Verification items for the finished model (mm, model axes). A direction names the side the tool comes from. Coordinates: 2 decimals unless noted, no trailing zeros. Order: outer loops, then holes, each group sorted by start corner. A loop starts at its lowest first (then second) coordinate and runs counter-clockwise, first axis right, second up. Notation, with made-up numbers: M 79,46.25 L 135,46.25 A13 cw 135,53.25 Z; hole C 13,23 d5. An arc over 180 degrees is marked long. Answer as a JSON object with one key per item and string values. Group by question number.
(1) Access from +Z, -Z, +X, -X, +Y, -Y to the whole of each face (thin tool, end or side, straight path). Record for faces 5 (the face through (-1, 0, 0)), 6 (the face through (-63, 3, 6.5)).
(2) Cross-section at A-A (y = 2.5). Enter the section's corners in (x, z).
(3) Material ranges on line 1 (Z direction, x = -65.5, y = 3.35); line 2 (Z direction, x = 56.5, y = 1.6), recorded low to high.
(4) Mould release check, pull along Z, two halves, no side actions. Record for faces 1 (the face through (63, 3, -6.5)), 2 (the face through (-1, 2, 24)), 3 (the face through (-53.5, 2.5, -0.1)), 4 (the face through (-1, 2, -24)): released by +Z, released by -Z, zero draft, split by the parting line, or undercut.
(5) Cross-section at B-B (z = -3). Enter the section's corners in (x, y), plus the area to 3 significant figures.
from build123d import *

# Parameters (mm, degrees)
SKETCH_1_W          = 172
SKETCH_1_H          = 48
EXTRUDE_1_DEPTH     = 5
CUT_EXTRUDE_1_DEPTH = 90.425947018


with BuildPart() as part:
    # 草图1 → 凸台-拉伸1 (new body)
    with BuildSketch(Plane(origin=(0, 0, 0), x_dir=(1, 0, 0), z_dir=(0, 1, 0))):
        Rectangle(SKETCH_1_W, SKETCH_1_H)
    extrude(amount=EXTRUDE_1_DEPTH)

    # 草图2 → 切除-拉伸1 (cut, through all)
    with BuildSketch(Plane(origin=(0, 5, 0), x_dir=(1, 0, 0), z_dir=(0, 1, 0))):
        with BuildLine():
            Line((66, -6.5), (60, -6.5))
            ThreePointArc((60, -6.5), (53.5, 0), (60, 6.5))
            Line((60, 6.5), (66, 6.5))
            ThreePointArc((66, 6.5), (72.5, 0), (66, -6.5))
        make_face()
        with BuildLine():
            Line((-66, 6.5), (-60, 6.5))
            ThreePointArc((-60, 6.5), (-53.5, 0), (-60, -6.5))
            Line((-60, -6.5), (-66, -6.5))
            ThreePointArc((-66, -6.5), (-72.5, 0), (-66, 6.5))
        make_face()
    extrude(amount=-CUT_EXTRUDE_1_DEPTH, mode=Mode.SUBTRACT)


solid = part.part
Taken from the geometry:
{
 "1": {"face 5": "+Z, -Z, +X, -X, -Y", "face 6": "+Y, -Y"},
 "2": {"outline": "M -86,-24 L 86,-24 L 86,24 L -86,24 Z; hole M -66,-6.5 L -60,-6.5 A6.5 ccw -60,6.5 L -66,6.5 A6.5 ccw Z; hole M 60,-6.5 L 66,-6.5 A6.5 ccw 66,6.5 L 60,6.5 A6.5 ccw Z"},
 "3": {"line 1": "z = -24 to -6.5, 6.5 to 24", "line 2": "z = -24 to -5.48, 5.48 to 24"},
 "4": {"face 1": "undercut", "face 2": "released by +Z", "face 3": "undercut", "face 4": "released by -Z"},
 "5": {"outline": "M -86,0 L -71.77,0 L -71.77,5 L -86,5 Z; M -54.23,0 L 54.23,0 L 54.23,5 L -54.23,5 Z; M 71.77,0 L 86,0 L 86,5 L 71.77,5 Z", "area": "685 mm²"}
}
